Geometry check sheet. Reference: the model listing, model coordinates, mm. Face numbers are marked on the shaded views. A direction names the side the tool comes from. Give positions to 0.01 mm unless a question says otherwise; leave off trailing zeros. Order: outer loops, then holes, each group sorted by start corner. A loop starts at its lowest first (then second) coordinate and runs counter-clockwise, first axis right, second up. Notation, with made-up numbers: M 42,48 L 78,48 A22 cw 78,68 Z; hole C 77,70.5 d10. An arc over 180 degrees is marked long. Answer as CSV lines item,"result".
from build123d import *

# Parameters (mm, degrees)
BOSS_EXTRUDE1_DEPTH = 5
BOSS_EXTRUDE2_DEPTH = 1
SKETCH5_R           = 3
BOSS_EXTRUDE3_DEPTH = 5
SKETCH6_R           = 2
CUT_EXTRUDE1_DEPTH  = 5
SKETCH7_R           = 6
SKETCH7_R_2         = 8
BOSS_EXTRUDE4_DEPTH = 8
SKETCH8_R           = 6
SKETCH8_R_2         = 4
CUT_EXTRUDE2_DEPTH  = 11
CUT_EXTRUDE3_DEPTH  = 1.4


with BuildPart() as part:
    # Sketch2 → Boss-Extrude1 (new body)
    with BuildSketch(Plane.XY):
        with BuildLine():
            Line((-20, 28), (20, 28))
            ThreePointArc((20, 28), (48, 0), (20, -28))
            Line((20, -28), (-20, -28))
            ThreePointArc((-20, -28), (-48, 0), (-20, 28))
        make_face()
    extrude(amount=BOSS_EXTRUDE1_DEPTH)

    # Sketch4 → Boss-Extrude2 (add)
    with BuildSketch(Plane.XY.offset(5)):
        with BuildLine():
            Line((-20, 25), (20, 25))
            ThreePointArc((20, 25), (45, 0), (20, -25))
            Line((20, -25), (-20, -25))
            ThreePointArc((-20, -25), (-45, 0), (-20, 25))
        make_face()
    extrude(amount=BOSS_EXTRUDE2_DEPTH)

    # Sketch5 → Boss-Extrude3 (add)
    with BuildSketch(Plane(origin=(0, 0, 0), x_dir=(-1, 0, 0), z_dir=(0, 0, -1))):
        with Locations((-20, 28)):
            Circle(SKETCH5_R)
        with Locations((20, 28)):
            Circle(SKETCH5_R)
        with Locations((-20, -28)):
            Circle(SKETCH5_R)
        with Locations((20, -28)):
            Circle(SKETCH5_R)
    extrude(amount=-BOSS_EXTRUDE3_DEPTH)

    # Sketch6 → Cut-Extrude1 (cut)
    with BuildSketch(Plane(origin=(0, 0, 0), x_dir=(-1, 0, 0), z_dir=(0, 0, -1))):
        with Locations((-20, 28)):
            Circle(SKETCH6_R)
        with Locations((20, 28)):
            Circle(SKETCH6_R)
        with Locations((-20, -28)):
            Circle(SKETCH6_R)
        with Locations((20, -28)):
            Circle(SKETCH6_R)
    extrude(amount=-CUT_EXTRUDE1_DEPTH, mode=Mode.SUBTRACT)

    # Sketch7 → Boss-Extrude4 (add)
    with BuildSketch(Plane(origin=(0, 0, 0), x_dir=(-1, 0, 0), z_dir=(0, 0, -1))):
        with Locations(Location((-20, 0, 0), (0, 0, 180))):
            Circle(SKETCH7_R)
        with Locations(Location((20, 0, 0), (0, 0, 180))):
            Circle(SKETCH7_R_2)
    extrude(amount=BOSS_EXTRUDE4_DEPTH)

    # Sketch8 → Cut-Extrude2 (cut)
    with BuildSketch(Plane.XY.offset(6)):
        with Locations((-20, 0)):
            Circle(SKETCH8_R)
        with Locations((20, 0)):
            Circle(SKETCH8_R_2)
    extrude(amount=-CUT_EXTRUDE2_DEPTH, mode=Mode.SUBTRACT)

    # Sketch9 → Cut-Extrude3 (cut, symmetric)
    with BuildSketch(Plane(origin=(0, 4, 0), x_dir=(1, 0, 0), z_dir=(0, 1, 0))):
        with BuildLine():
            Line((18.5, -7.970089987), (18.5, 1.6))
            ThreePointArc((18.5, 1.6), (20, 3.1), (21.5, 1.6))
            Line((21.5, 1.6), (21.5, -7.970089987))
            ThreePointArc((21.5, -7.970089987), (20, -9.470089987), (18.5, -7.970089987))
        make_face()
    extrude(amount=CUT_EXTRUDE3_DEPTH, both=True, mode=Mode.SUBTRACT)


solid = part.part
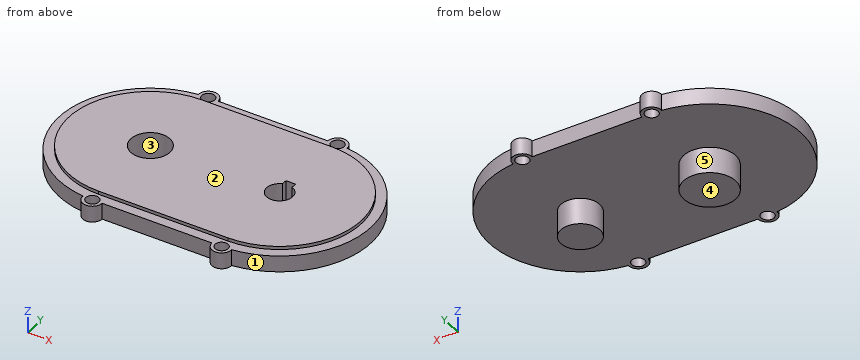
(1) Section check A-A on z = 3.75. Enter the section's corners in (x, y).
The answers:
outline,"M -23,-27.84 A3 ccw long -17,-28 L 17,-28 A3 ccw long 23,-27.84 A28 ccw 23,27.84 A3 ccw long 17,28 L -17,28 A3 ccw long -23,27.84 A28 ccw Z; hole C -20,0 d12; hole C -20,-28 d4; hole C -20,28 d4; hole C 20,-28 d4; hole C 20,28 d4; hole M 18.5,3.71 A4 ccw long 21.5,3.71 L 21.5,5.4 L 18.5,5.4 Z"
(2) Section check D-D on x = -16. Enter the section's corners in (y, z).
The answers:
outline,"M -28,0 L -6.93,0 L -6.93,-8 L 6.93,-8 L 6.93,0 L 28,0 L 28,5 L 25,5 L 25,6 L 4.47,6 L 4.47,-5 L -4.47,-5 L -4.47,6 L -25,6 L -25,5 L -28,5 Z"
(3) Gauge pin test, flat ends, axial feed: P1, Ø6, axis at y = -6, z = -1, coming from the -X side; P2, Ø2, axis at x = 29.5, z = -2.5, coming from the +Y side; P3, Ø2, axis at y = -11.5, z = -0.5, coming from the -X side; P4, Ø1.1, axis at x = -3, z = 5.5, coming from the +Y side. Record the tip position at first contact, or that the pin passes through.
The answers:
P1,"stops at x = -47.82"
P2,"passes through"
P3,"stops at x = -45.9"
P4,"stops at y = 28"
(4) Section check C-C on y = -15.5. Enter the section's corners in (x, z).
The answers:
outline,"M -43.32,0 L 43.32,0 L 43.32,5 L 39.62,5 L 39.62,6 L -39.62,6 L -39.62,5 L -43.32,5 Z"
(5) Material ranges on line 1 (Y direction, x = -20, z = 2.55); line 2 (Y direction, x = 20, z = 3.8); line 3 (Y direction, x = 20, z = -2.5), recorded low to high.
The answers:
line 1,"y = -31 to -30, -26 to -6, 6 to 26, 30 to 31"
line 2,"y = -31 to -30, -26 to -4, 5.4 to 26, 30 to 31"
line 3,"y = -6 to -4, 5.4 to 6"
(6) Section check B-B on x = 7.5. Enter the section's corners in (y, z).
The answers:
outline,"M -28,0 L 28,0 L 28,5 L 25,5 L 25,6 L -25,6 L -25,5 L -28,5 Z"
(7) Draft check along X on the marked faces 1, 2 and 3. Enter one of: +X half, -X half, draft (parallel to the pull), parting line (faces both ways), or undercut.
The answers:
face 1,"+X half"
face 2,"draft"
face 3,"undercut"
(8) Tool access check on the marked faces 4 and 5. Record the directions out of +Z, -Z, +X, -X, +Y, -Y that give a thin tool (end or side, any length) a straight path to the whole face; none if there is none.
The answers:
face 4,"-Z, +X, -X, +Y, -Y"
face 5,"-Z"
